Drawing for the job (mm, zero at the part's lowest x, y, z). A direction names the side the tool comes from. Give positions to 0.01 mm unless a question says otherwise; leave off trailing zeros. Loops run counter-clockwise (first coordinate to the right, second up) from the corner with the lowest first, then second, coordinate; pieces in that order, holes last. Notation, with made-up numbers: M 13,58.25 L 66,58.25 A20 cw 66,64.25 Z; hole C 2,77.5 d5. An arc over 180 degrees is marked long. Use CSV: the item, a comma, the result in double quotes. Start each with the question number.
(1) Slice it at B-B on x = 7. List the corners of the cut face in (y, z), and give its area (3 significant figures).
(2) Tool access for the marked faces 1, 2 and 3: list every direction of +Z, -Z, +X, -X, +Y, -Y with a clear straight run to the whole face (end or side of a thin tool).
(3) Slice it at A-A on x = 53. List the corners of the cut face in (y, z), and give its area (3 significant figures).
(4) Flat gauge pins, fed straight in: P1, Ø3, axis at x = 64, y = 6, coming from the -Z side; P2, Ø5, axis at x = 54, z = 2.5, coming from the +Y side; P3, Ø6, axis at x = 45, y = 8, coming from the +Z side. Where does each tip first touch, or does it go through?
(5) Wall check: line 1 along Z through (x, y) = (4.5, 1.5); line 2 along X through (y, z) = (2.5, 3.75) (1 decimal); line 3 along Y through (x, z) = (11, 5.25) (1 decimal). Give the ranges that are in metal, low to high. Write a range as from..to.
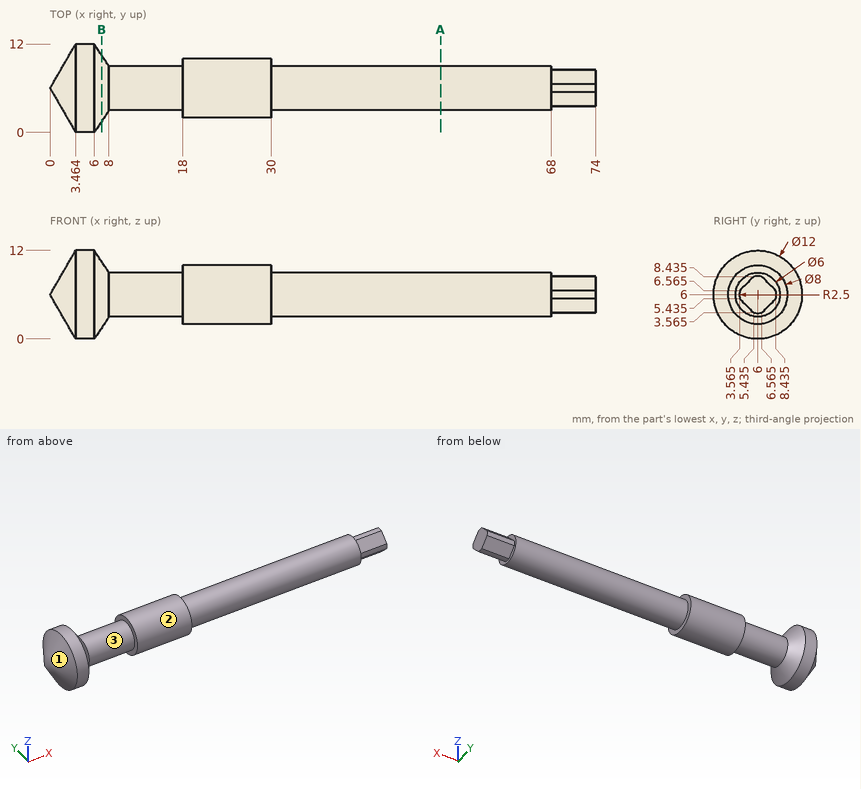
Reply:
1,outline,"C 6,6 d9"
1,area,"63.6 mm^2"
2,face 1,"-X"
2,face 2,"+X"
2,face 3,"none"
3,outline,"C 6,6 d6"
3,area,"28.3 mm^2"
4,P1,"stops at z = 3"
4,P2,"stops at y = 8.83"
4,P3,"stops at z = 9"
5,line 1,"z = 2.03..9.97"
5,line 2,"x = 2.4..7.2"
5,line 3,"y = 3.1..8.9"
